Can you work these out from the drawing? Everything is in mm from the part's minimum corner. A direction names the side the tool comes from. Give positions to 0.01 mm unless a question says otherwise; leave off trailing zeros. Order: outer loops, then holes, each group sorted by start corner. A loop starts at its lowest first (then second) coordinate and runs counter-clockwise, first axis right, second up. Notation, with made-up numbers: (20, 14) -> (42, 14) arc R20 cw to (42, 51) -> close; hole circle Ø2 at (1, 85.25). An arc over 180 degrees is marked (long way). One line per item, written item: value.
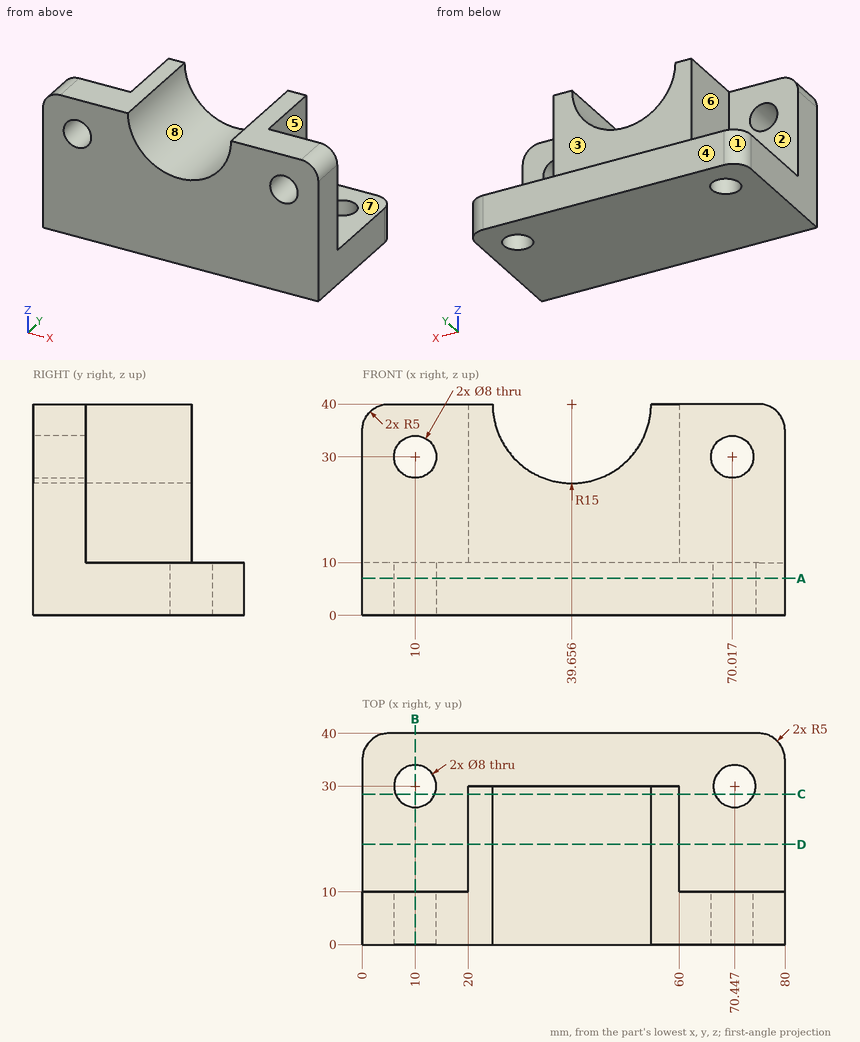
1) Suppose I cut it at B-B, the plane x = 10. Write out the boundary of the cut face in (y, z), then the cut area to 3 significant figures.
Answer below:
outline: (0, 0) -> (26, 0) -> (26, 10) -> (10, 10) -> (10, 26) -> (0, 26) -> close; (0, 34) -> (10, 34) -> (10, 40) -> (0, 40) -> close; (34, 0) -> (40, 0) -> (40, 10) -> (34, 10) -> close
area: 540 mm2
2) We'd pull the mould along X, two halves only. Please class the marked faces 6, 7 and 8: +X half, -X half, draft (parallel to the pull), parting line (faces both ways), or undercut.
Answer below:
face 6: -X half
face 7: draft
face 8: undercut
3) If I drill on line 1 along X through (y, z) = (2.5, 30) (1 decimal); line 2 along Y through (x, z) = (10, 5.5); line 3 along Y through (x, z) = (3, 16), over which ranges is the centre line in solid material (lowest first)?
Answer below:
line 1: x = 0 to 6, 14 to 28.5, 50.8 to 66, 74 to 80
line 2: y = 0 to 26, 34 to 40
line 3: y = 0 to 10
4) Suppose I cut it at D-D, the plane y = 19. Write out the boundary of the cut face in (x, z), then the cut area to 3 significant figures.
Answer below:
outline: (0, 0) -> (80, 0) -> (80, 10) -> (60, 10) -> (60, 40) -> (54.66, 40) arc R15 cw to (24.66, 40) -> (20, 40) -> (20, 10) -> (0, 10) -> close
area: 1,650 mm2
5) For the marked faces 1, 2, 3, 4 and 5, which set-ups out of +Z, -Z, +X, -X, +Y, -Y let a thin tool reach every point of the face, with its end or its side?
Answer below:
face 1: +Z, -Z, -X, +Y
face 2: +Z, -X, +Y
face 3: +Z, +X, -X, +Y
face 4: +Z, -Z, +X, -X, +Y
face 5: +Z, +X, +Y
6) For P1, Ø4, axis at x = 53, y = 31, coming from the -Z side; P2, Ø12, axis at y = 29.5, z = 35, coming from the -X side; P3, Ø6, axis at y = 30.5, z = 30.5, coming from the +X side; P4, Ø15, axis at x = 42.5, z = 19.5, coming from the +Y side, each with a flat end and sliding along its axis, tell me the tip position at first contact or that it passes through.
Answer below:
P1: stops at z = 0
P2: stops at x = 20
P3: stops at x = 60
P4: stops at y = 30
7) Suppose I cut it at C-C, the plane y = 28.5. Write out the boundary of the cut face in (x, z) (1 decimal).
Answer below:
outline: (0, 0) -> (6.3, 0) -> (6.3, 10) -> (0, 10) -> close; (13.7, 0) -> (66.7, 0) -> (66.7, 10) -> (60, 10) -> (60, 40) -> (54.7, 40) arc R15 cw to (24.7, 40) -> (20, 40) -> (20, 10) -> (13.7, 10) -> close; (74.2, 0) -> (80, 0) -> (80, 10) -> (74.2, 10) -> close
8) Suppose I cut it at A-A, the plane z = 7. Write out the boundary of the cut face in (x, y).
Answer below:
outline: (0, 0) -> (80, 0) -> (80, 35) arc R5 ccw to (75, 40) -> (5, 40) arc R5 ccw to (0, 35) -> close; hole circle Ø8 at (10, 30); hole circle Ø8 at (70.45, 30)
